from build123d import *

# Parameters (mm, degrees)
FILLET1_R = 0.6
FILLET2_R = 0.6


with BuildPart() as part:
    # Sketch1 → Revolve1 (revolve)
    with BuildSketch(Plane.XY, mode=Mode.PRIVATE) as revolve1_sk:
        Polygon((0, 22.5), (12, 22.5), (12, 25), (11.45, 25), (11.45, 31.75), (12, 31.75), (12, 34), (0, 34), (0, 31.75), (0.55, 31.75), (0.55, 25), (0, 25), align=None)
    revolve(revolve1_sk.sketch.rotate(Axis((0, 0, 0), (1, 0, 0)), 90), axis=Axis((0, 0, 0), (1, 0, 0)))

    # Fillet1
    fillet1_edges = [part.edges().sort_by_distance(p)[0] for p in [
        (0, 0, -34),
        (12, 0, -34),
    ]]
    fillet(fillet1_edges, radius=FILLET1_R)

    # Fillet2
    fillet2_edges = [part.edges().sort_by_distance(p)[0] for p in [
        (12, 0, -22.5),
        (0, 0, -22.5),
    ]]
    fillet(fillet2_edges, radius=FILLET2_R)


solid = part.part
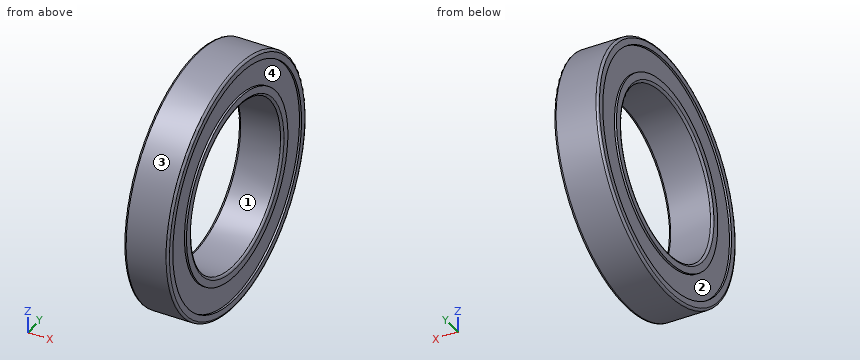
The listing builds one solid part. Answer for the finished solid, in the listing's coordinates (mm). Face numbers are marked on the shaded views. A direction names the side the tool comes from. Give positions to 0.01 mm unless a question says otherwise; leave off trailing zeros. Order: outer loops, then holes, each group sorted by start corner. A loop starts at its lowest first (then second) coordinate and runs counter-clockwise, first axis right, second up. Notation, with made-up numbers: (30.25, 2.25) - (79.25, 2.25) arc R31 ccw to (79.25, 32.25) - close; hole circle Ø3 at (17.5, 33.5). An arc over 180 degrees is marked (long way). One line per item, written item: value. Start each with the question number.
1) The mould has two halves that part along Y. Classify the marked faces 3 and 4: released by +Y, released by -Y, zero draft, split by the parting line, or undercut.
2) A cutting plane is placed at C-C on x = 1.5. Give the vertices of the cut face in (y, z), then the cut area to 3 significant figures.
3) A tool of negligible diameter and unlimited length cuts with its end or side. For the marked faces 1 and 2, from which of +Z, -Z, +X, -X, +Y, -Y can it reach the whole face along a straight path? Write none if from no direction.
4) Given pin 1 Ø5 at (x, z) = (10, 20.5) entering from -Y; pin 2 Ø3 at (y, z) = (-16.5, -22) entering from -X; pin 3 Ø1 at (x, z) = (6.5, 10) entering from -Y, each flat-ended and moving along its own axis, determine where each tip first touches the part or whether it passes through.
5) Find the intervals of material crossed by L1, parallel to Y at x = 7.25, z = 0; L2, parallel to Z at x = 11.5, y = 9; L3, parallel to X at y = 26.5, z = -3, in increasing order.
Answer sheet:
1. face 3: split by the parting line
1. face 4: undercut
2. outline: circle Ø68 at (0, 0); hole circle Ø45 at (0, 0)
2. area: 2,040 mm2
3. face 1: +X, -X
3. face 2: -X
4. pin 1: stops at y = -28.84
4. pin 2: stops at x = 0.55
4. pin 3: stops at y = -32.65
5. L1: y = -34 to -22.5, 22.5 to 34
5. L2: z = -32.78 to -30.45, -23.32 to -20.63, 20.63 to 23.32, 30.45 to 32.78
5. L3: x = 0.55 to 11.45
